Check sheet for the drawn part. Datum: minimum x, y, z corner. Units: mm. Coordinates: 2 decimals unless noted, no trailing zeros. Loops run counter-clockwise (first coordinate to the right, second up) from the corner with the lowest first, then second, coordinate; pieces in that order, holes last.
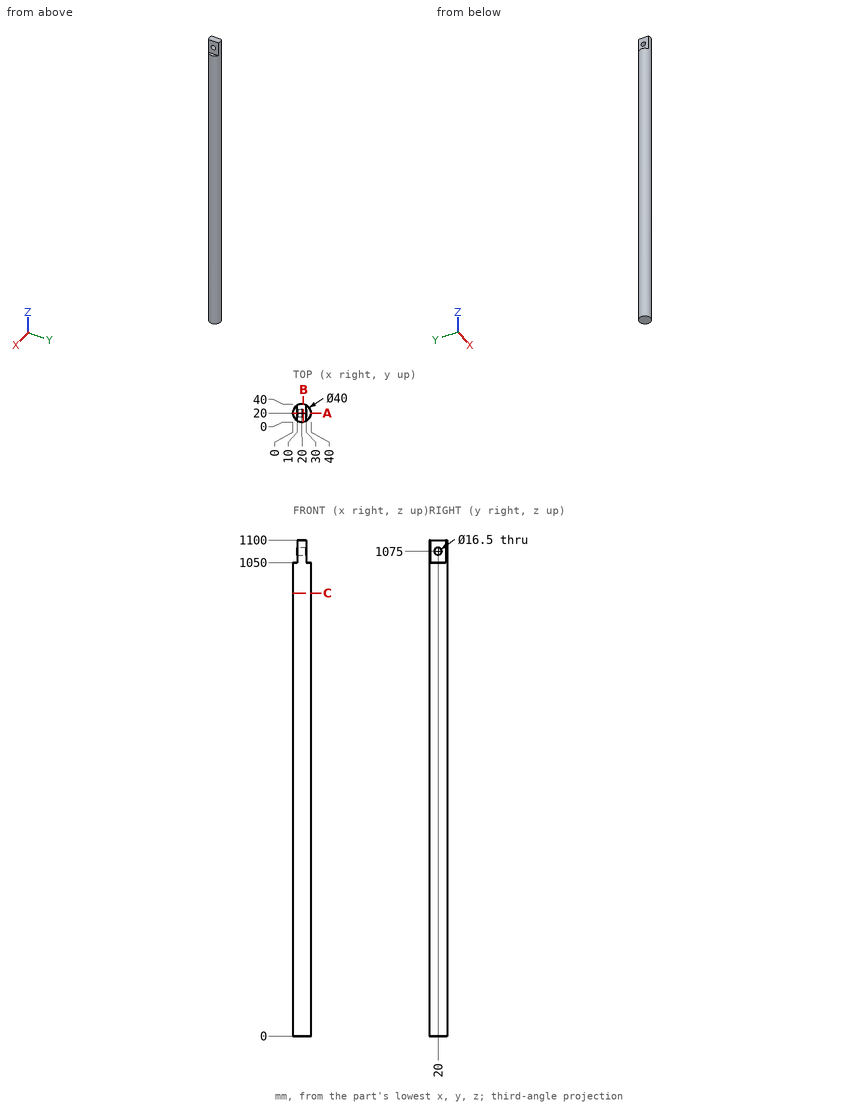
1) Depth check by flat-ended pin: pin 1 (3 mm diameter, centred on x = 31, z = 669, fed in from -Y); pin 2 (12 mm diameter, centred on y = 5.5, z = 844, fed in from +X); pin 3 (10.5 mm diameter, centred on y = 12, z = 1063, fed in from +X); pin 4 (2 mm diameter, centred on x = 4.5, y = 35.5, fed in from +Z). Enter the tip coordinate at first touch or a pass-through.
Answer sheet:
pin 1: stops at y = 2.4
pin 2: stops at x = 38.1
pin 3: stops at x = 30
pin 4: passes through
2) Section check B-B on x = 23. Enter the section's corners in (y, z), plus the area to 3 significant figures.
Answer sheet:
outline: (0.23, 0) - (39.77, 0) - (39.77, 1100) - (0.23, 1100) - close; hole circle Ø16.5 at (20, 1075)
area: 43,300 mm2
3) Section check A-A on y = 20. Enter the section's corners in (x, z), plus the area to 3 significant figures.
Answer sheet:
outline: (0, 0) - (40, 0) - (40, 1050) - (30, 1050) - (30, 1066.75) - (10, 1066.75) - (10, 1050) - (0, 1050) - close; (10, 1083.25) - (30, 1083.25) - (30, 1100) - (10, 1100) - close
area: 42,700 mm2
4) Scan lines: line 1 (Y direction, x = 20, z = 1075); line 2 (Z direction, x = 14, y = 20); line 3 (X direction, y = 19, z = 521.5). Record each from-to range of solid material in increasing order.
Answer sheet:
line 1: y = 0 to 11.75, 28.25 to 40
line 2: z = 0 to 1066.75, 1083.25 to 1100
line 3: x = 0.03 to 39.97
5) Section check C-C on z = 982. Enter the section's corners in (x, y), plus the area to 3 significant figures.
Answer sheet:
outline: circle Ø40 at (20, 20)
area: 1,260 mm2
